CAD build for the part. Positions are in the model's coordinates, mm. A direction names the side the tool comes from. Give positions to 0.01 mm unless a question says otherwise; leave off trailing zeros. Loops run counter-clockwise (first coordinate to the right, second up) from the corner with the lowest first, then second, coordinate; pieces in that order, holes last. Notation, with made-up numbers: M -38,89 L -29,89 A15 cw -29,108 Z; hole C -36,-14 d6. An arc over 180 degrees is marked long. Answer as CSV lines item,"result".
from build123d import *

# Parameters (mm, degrees)
SKETCH2_R             = 1.5
CUT_EXTRUDE1_DEPTH    = 3
M4_TAPPED_HOLE1_D     = 3.3
M4_TAPPED_HOLE1_DEPTH = 8
M4_TAPPED_HOLE1_TIP   = 0.991420021
CHAMFER1_SIZE         = 0.375
CHAMFER2_SIZE         = 1


with BuildPart() as part:
    # Sketch1 → Revolve1 (revolve)
    with BuildSketch(Plane(origin=(0, 0, 0), x_dir=(1, 0, 0), z_dir=(0, 1, 0))):
        Polygon((25, 0), (42, 0), (42, 3), (45, 3), (45, 11), (25, 11), align=None)
    revolve(axis=Axis((0, 0, 0), (0, 0, -1)))

    # Sketch2 → Cut-Extrude1 (cut)
    with BuildSketch(Plane(origin=(0, 0, -11), x_dir=(-1, 0, 0), z_dir=(0, 0, -1))):
        with Locations((0, -37)):
            Circle(SKETCH2_R)
        with Locations((-32.04293994, -18.5)):
            Circle(SKETCH2_R)
        with Locations((-32.04293994, 18.5)):
            Circle(SKETCH2_R)
        with Locations((0, 37)):
            Circle(SKETCH2_R)
        with Locations((32.04293994, 18.5)):
            Circle(SKETCH2_R)
        with Locations((32.04293994, -18.5)):
            Circle(SKETCH2_R)
    extrude(amount=-CUT_EXTRUDE1_DEPTH, mode=Mode.SUBTRACT)

    # M4 Tapped Hole1
    with Locations(Plane(origin=(0, 0, -11), x_dir=(-1, 0, 0), z_dir=(0, 0, -1))):
        with Locations((0, -37), (-32.04293994, -18.5), (-32.04293994, 18.5), (0, 37), (32.04293994, -18.5), (32.04293994, 18.5)):
            Hole(M4_TAPPED_HOLE1_D / 2, depth=M4_TAPPED_HOLE1_DEPTH)
            with Locations((0, 0, -(M4_TAPPED_HOLE1_DEPTH + M4_TAPPED_HOLE1_TIP / 2))):  # 118° drill point
                Cone(0, M4_TAPPED_HOLE1_D / 2, M4_TAPPED_HOLE1_TIP, mode=Mode.SUBTRACT)

    # Chamfer1
    chamfer1_edges = [part.edges().sort_by_distance(p)[0] for p in [
        (-33.69293994, 18.5, -11),
        (-33.69293994, -18.5, -11),
        (-1.65, 37, -11),
        (30.39293994, 18.5, -11),
        (30.39293994, -18.5, -11),
        (-1.65, -37, -11),
    ]]
    chamfer(chamfer1_edges, length=CHAMFER1_SIZE)

    # Chamfer2
    chamfer2_edges = [part.edges().sort_by_distance(p)[0] for p in [
        (-25, 0, -11),
        (-45, 0, -11),
        (-42, 0, 0),
    ]]
    chamfer(chamfer2_edges, length=CHAMFER2_SIZE)


solid = part.part
1) Drill centre lines: line 1 (Y direction, x = 0, z = -8); line 2 (X direction, y = -18.5, z = -9); line 3 (X direction, y = -17, z = -6). Where is each one in solid material? Low to high. Write a range as from..to.
Answer below:
line 1,"y = -45..-38.65, -35.35..-25, 25..35.35, 38.65..45"
line 2,"x = -41.02..-33.69, -30.39..-16.82, 16.82..30.39, 33.69..41.02"
line 3,"x = -41.67..-32.73, -31.36..-18.33, 18.33..31.36, 32.73..41.67"
2) Band-saw the part on A-A on y = 0. Give the cut face in (x, z).
Answer below:
outline,"M -45,-10 L -44,-11 L -26,-11 L -25,-10 L -25,0 L -41,0 L -42,-1 L -42,-3 L -45,-3 Z; M 25,-10 L 26,-11 L 44,-11 L 45,-10 L 45,-3 L 42,-3 L 42,-1 L 41,0 L 25,0 Z"
3) Band-saw the part on B-B on z = -8.25. Give the cut face in (x, y), and give its area (3 significant figures).
Answer below:
outline,"C 0,0 d90; hole C -32.04,-18.5 d3.3; hole C -32.04,18.5 d3.3; hole C 0,0 d50; hole C 0,-37 d3.3; hole C 0,37 d3.3; hole C 32.04,-18.5 d3.3; hole C 32.04,18.5 d3.3"
area,"4,350 mm^2"
4) Mould opens along X. For faces 1 (the face through (0.89, -35.61, -6.76)), 2 (the face through (19, 19, -11)), 3 (the face through (40.06, -12.62, -2.01)) say: +X half, -X half, draft (parallel to the pull), parting line (faces both ways), or undercut.
Answer below:
face 1,"undercut"
face 2,"draft"
face 3,"parting line"
5) Flat gauge pins, fed straight in: pin 1 (2 mm diameter, centred on x = -32.04, y = 18.5, fed in from -Z); pin 2 (5 mm diameter, centred on x = -32.5, z = -8, fed in from -Y); pin 3 (2.5 mm diameter, centred on x = 32.04, y = -18.5, fed in from +Z); pin 4 (1.5 mm diameter, centred on y = 20, z = -6, fed in from +X). Where does each tip first touch, or does it go through?
Answer below:
pin 1,"stops at z = -2.61"
pin 2,"stops at y = -33.54"
pin 3,"stops at z = 0"
pin 4,"stops at x = 40.67"
6) Which spindle directions (+Z, -Z, +X, -X, +Y, -Y) get a long thin tool onto all of the face, cutting with end or side? Do faces 4 (the face through (20.765, 39.923, -6.549)), 5 (the face through (30.83, -17.38, -6.76)). Say none if no direction does.
Answer below:
face 4,"+Z, -Z"
face 5,"-Z"
